```python
from build123d import *

# Parameters (mm, degrees)
SKETCH1_R           = 10
BOSS_EXTRUDE1_DEPTH = 15


with BuildPart() as part:
    # Sketch1 → Boss-Extrude1 (new body)
    with BuildSketch(Plane(origin=(0, 0, 0), x_dir=(1, 0, 0), z_dir=(0, 1, 0))):
        with BuildLine():
            Line((-20, 0), (-20, 300))
            ThreePointArc((-20, 300), (0, 320), (20, 300))
            Line((20, 300), (20, 0))
            ThreePointArc((20, 0), (0, -20), (-20, 0))
        make_face()
        with Locations(Location((0, 300, 0), (0, 0, 270))):
            Circle(SKETCH1_R, mode=Mode.SUBTRACT)
        with Locations(Location((0, 0, 0), (0, 0, 270))):
            Circle(SKETCH1_R, mode=Mode.SUBTRACT)
    extrude(amount=BOSS_EXTRUDE1_DEPTH)


solid = part.part
```
Can you work these out from the model? Positions are in its coordinate system, mm. Round coordinates to 2 decimals unless told otherwise and drop trailing zeros. Loops run counter-clockwise (first coordinate to the right, second up) from the corner with the lowest first, then second, coordinate; pieces in that order, holes last. Notation, with made-up numbers: (-26, -23) -> (-9, -23) arc R11 cw to (-9, -15) -> close; hole circle Ø11 at (74.25, 39). An arc over 180 degrees is marked (long way). Answer in a Markdown table with one row per item.
Item 1: If I drill on probe 1 along Z at (x, y) = (-1, 2.5); probe 2 along Z at (x, y) = (-3.5, 9.5); probe 3 along X at (y, z) = (5, -300), over which ranges is the centre line in solid material (lowest first)?
Answer block:
| item | result |
|---|---|
| probe 1 | -319.97 to -309.95, -290.05 to -9.95, 9.95 to 19.97 |
| probe 2 | -319.69 to -309.37, -290.63 to -9.37, 9.37 to 19.69 |
| probe 3 | -20 to -10, 10 to 20 |
Item 2: Suppose I cut it at B-B, the plane y = 12.5. List the corners of the cut face in (x, z) for me, plus the area to 3 significant figures.
Answer block:
| item | result |
|---|---|
| outline | (-20, -300) arc R20 ccw to (20, -300) -> (20, 0) arc R20 ccw to (-20, 0) -> close; hole circle Ø20 at (0, -300); hole circle Ø20 at (0, 0) |
| area | 12,600 mm² |
Item 3: Suppose I cut it at C-C, the plane x = 17. List the corners of the cut face in (y, z) for me, plus the area to 3 significant figures.
Answer block:
| item | result |
|---|---|
| outline | (0, -310.54) -> (15, -310.54) -> (15, 10.54) -> (0, 10.54) -> close |
| area | 4,820 mm² |
Item 4: Will these pins go through, and if not, where does the flat tip stop? P1, Ø1.5, axis at x = 1.5, y = 13, coming from the +Z side; P2, Ø1.5, axis at x = 4.5, y = 13, coming from the -Z side; P3, Ø2, axis at x = -6.5, y = 3.5, coming from the +Z side.
Answer block:
| item | result |
|---|---|
| P1 | z = 19.99 |
| P2 | z = -319.65 |
| P3 | z = 19.23 |
Item 5: We'd pull the mould along Z, two halves only. Please class faces 1 (the cylindrical face through (0, 7, -310)), 2 (the flat face through (0, 15, -152)), 3 (the cylindrical face through (0, 7, -320)): released by +Z, released by -Z, zero draft, split by the parting line, or undercut.
Answer block:
| item | result |
|---|---|
| face 1 | undercut |
| face 2 | zero draft |
| face 3 | released by -Z |
Item 6: Suppose I cut it at A-A, the plane x = 0. List the corners of the cut face in (y, z) for me.
Answer block:
| item | result |
|---|---|
| outline | (0, -320) -> (15, -320) -> (15, -310) -> (0, -310) -> close; (0, -290) -> (15, -290) -> (15, -10) -> (0, -10) -> close; (0, 10) -> (15, 10) -> (15, 20) -> (0, 20) -> close |
